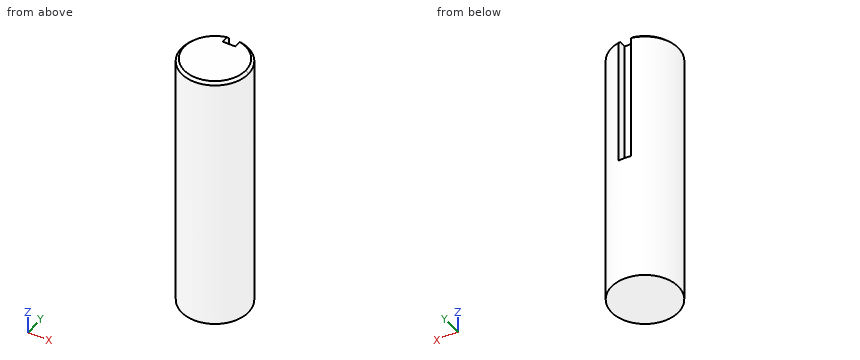
```python
from build123d import *

# Parameters (mm, degrees)
SHAFT_PROFILE_75_R      = 37.5
SHAFT_BODY_75X294_DEPTH = 294
KEYWAY_START            = -147
KEYWAY_CUT_14X147_DEPTH = 147
END_CHAMFER_3X45_SIZE   = 3


with BuildPart() as part:
    # Shaft Profile Ø75 → Shaft Body Ø75x294 (new body)
    with BuildSketch(Plane.XY):
        Circle(SHAFT_PROFILE_75_R)
    extrude(amount=SHAFT_BODY_75X294_DEPTH)

    # Keyway Profile 14 wide → Keyway Cut 14x147 (cut)
    with BuildSketch(Plane.XY.offset(294).offset(KEYWAY_START)):
        with BuildLine():
            Line((-7, 25.84087404), (7, 25.84087404))
            Line((7, 25.84087404), (7, 36.84087404))
            ThreePointArc((7, 36.84087404), (0, 37.5), (-7, 36.84087404))
            Line((-7, 36.84087404), (-7, 25.84087404))
        make_face()
    extrude(amount=KEYWAY_CUT_14X147_DEPTH, mode=Mode.SUBTRACT)

    # End Chamfer 3x45°
    end_chamfer_3x45_edges = [part.edges().sort_by_distance(p)[0] for p in [
        (-23.913908087, -28.885550021, 294),
    ]]
    chamfer(end_chamfer_3x45_edges, length=END_CHAMFER_3X45_SIZE)


solid = part.part
```
The listing builds one solid part. Answer for the finished solid, in the listing's coordinates (mm). Coordinates: 2 decimals unless noted, no trailing zeros. Order: outer loops, then holes, each group sorted by start corner. A loop starts at its lowest first (then second) coordinate and runs counter-clockwise, first axis right, second up. Notation, with made-up numbers: M 52,-25 L 66,-25 A23 cw 66,4 Z; hole C -38.5,62 d10. An arc over 180 degrees is marked long. Answer as a JSON object with one key per item and string values. Group by question number.
1. Straight lines are drawn through the part: line 1 (X direction, y = 26, z = 192.5); line 2 (Y direction, x = 0.5, z = 255); line 3 (X direction, y = 34, z = 241). For each, find the intervals that lie inside material, in ascending order.
2. Section A-A on x = 0 is taken. Write down the section's boundary in (y, z).
3. Section C-C on z = 207 is taken. Write down the section's boundary in (x, y), then the cut area to 3 significant figures.
4. Section B-B on z = 103.5 is taken. Write down the section's boundary in (x, y).
5. Flat-ended cylindrical pins translate along their axes: P1, Ø2, axis at x = 7, y = 19, coming from the -Z side; P2, Ø1, axis at x = -26.5, z = 200, coming from the +Y side; P3, Ø7, axis at x = 2.5, z = 195.5, coming from the +Y side; P4, Ø6, axis at y = -13.5, z = 195, coming from the +X side. Find the tip coordinate at first contact, or state that the pin passes through.
Values follow:
{
 "1": {"line 1": "-27.02 to -7, 7 to 27.02", "line 2": "-37.5 to 25.84", "line 3": "-15.82 to -7, 7 to 15.82"},
 "2": {"outline": "M -37.5,0 L 37.5,0 L 37.5,147 L 25.84,147 L 25.84,294 L -34.5,294 L -37.5,291 Z"},
 "3": {"outline": "M -7,25.84 L -7,36.84 A37.5 ccw long 7,36.84 L 7,25.84 Z", "area": "4,260 mm2"},
 "4": {"outline": "C 0,0 d75"},
 "5": {"P1": "z = 0", "P2": "y = 27.02", "P3": "y = 25.84", "P4": "x = 36"}
}
